Part model, mm, in its own coordinate system. Face numbers are marked on the shaded views. A direction names the side the tool comes from. Coordinates: 2 decimals unless noted, no trailing zeros. Loops run counter-clockwise (first coordinate to the right, second up) from the corner with the lowest first, then second, coordinate; pieces in that order, holes last.
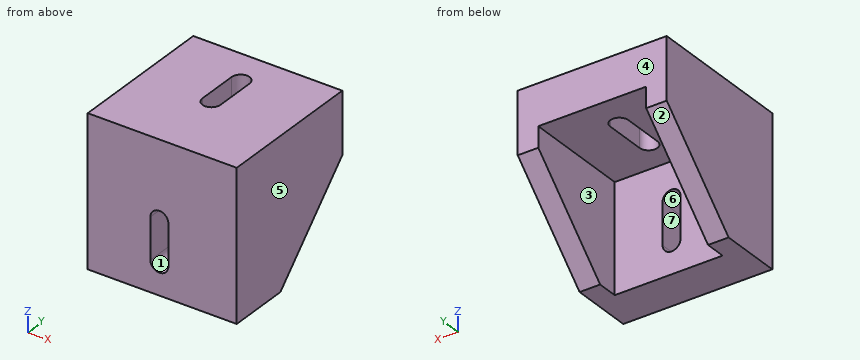
```python
from build123d import *

# Parameters (mm, degrees)
BASE_PLATE_SKETCH_W    = 29
BASE_PLATE_SKETCH_H    = 29
BASE_PLATE_8MM_DEPTH   = 8
BASE_SLOT_3_5MM_DEPTH  = 8
UPRIGHT_WALL_SKETCH_W  = 29
UPRIGHT_WALL_SKETCH_H  = 21
UPRIGHT_WALL_8MM_DEPTH = 8
WALL_SLOT_3_5MM_DEPTH  = 8
SIDE_BOSS_A_4MM_DEPTH  = 4
SIDE_BOSS_B_4MM_DEPTH  = 4


with BuildPart() as part:
    # Base Plate Sketch → Base Plate 8mm (new body)
    with BuildSketch(Plane.XY):
        with Locations((14.5, 14.5)):
            Rectangle(BASE_PLATE_SKETCH_W, BASE_PLATE_SKETCH_H)
    extrude(amount=BASE_PLATE_8MM_DEPTH)

    # Base Slot Sketch → Base Slot 3.5mm (cut)
    with BuildSketch(Plane.XY.offset(8)):
        with BuildLine():
            Line((12.234144505, 22.262653084), (12.234144505, 14.262653084))
            ThreePointArc((12.234144505, 14.262653084), (13.984144505, 12.512653084), (15.734144505, 14.262653084))
            Line((15.734144505, 14.262653084), (15.734144505, 22.262653084))
            ThreePointArc((15.734144505, 22.262653084), (13.984144505, 24.012653084), (12.234144505, 22.262653084))
        make_face()
    extrude(amount=-BASE_SLOT_3_5MM_DEPTH, mode=Mode.SUBTRACT)

    # Upright Wall Sketch → Upright Wall 8mm (add)
    with BuildSketch(Plane.XZ):
        with Locations((14.5, -10.5)):
            Rectangle(UPRIGHT_WALL_SKETCH_W, UPRIGHT_WALL_SKETCH_H)
    extrude(amount=-UPRIGHT_WALL_8MM_DEPTH)

    # Wall Slot Sketch → Wall Slot 3.5mm (cut)
    with BuildSketch(Plane(origin=(0, 8, 0), x_dir=(1, 0, 0), z_dir=(0, 1, 0))):
        with BuildLine():
            Line((12.192184218, 15), (12.192184218, 7))
            ThreePointArc((12.192184218, 7), (13.942184218, 5.25), (15.692184218, 7))
            Line((15.692184218, 7), (15.692184218, 15))
            ThreePointArc((15.692184218, 15), (13.942184218, 16.75), (12.192184218, 15))
        make_face()
    extrude(amount=-WALL_SLOT_3_5MM_DEPTH, mode=Mode.SUBTRACT)

    # Side Boss A Sketch → Side Boss A 4mm (add)
    with BuildSketch(Plane(origin=(29, 0, 0), x_dir=(0, 0, -1), z_dir=(1, 0, 0))):
        Polygon((0, 29), (4, 29), (21, 12), (21, 8), (0, 8), align=None)
    extrude(amount=-SIDE_BOSS_A_4MM_DEPTH)

    # Side Boss B Sketch → Side Boss B 4mm (add)
    with BuildSketch(Plane.ZY):
        Polygon((0, 29), (-4, 29), (-21, 12), (-21, 8), (0, 8), align=None)
    extrude(amount=-SIDE_BOSS_B_4MM_DEPTH)


solid = part.part
```
Q1. Probe line 1 (X direction, y = 2.75, z = -10.5); line 2 (X direction, y = 14.5, z = -15); line 3 (Z direction, x = 23.5, y = 22). List the from-to ranges inside material, lowest first.
Q2. Saw through at A-A (z = -14). List the corners of the cut face in (x, y).
Q3. Saw through at B-B (y = 17). List the corners of the cut face in (x, z), plus the area to 3 significant figures.
Q4. Saw through at D-D (x = 12.75). List the corners of the cut face in (y, z), plus the area to 3 significant figures.
Q5. Tool access for the marked faces 1, 2 and 3: list every direction of +Z, -Z, +X, -X, +Y, -Y with a clear straight run to the whole face (end or side of a thin tool).
Q6. Drop flat-ended pins along their axis: P1, Ø5, axis at x = 16, y = 24.5, coming from the -Z side; P2, Ø4, axis at x = 21.5, z = -13.5, coming from the +Y side. Give the stop position or say it passes through.
Q7. Mould opens along X. For the marked faces 4, 5, 6 and 7 say: released by +X, released by -X, zero draft, split by the parting line, or undercut.
Q8. Saw through at C-C (z = 0.75). List the corners of the cut face in (x, y).
Checked values:
1. line 1: x = 0 to 12.19, 15.69 to 29
1. line 2: x = 0 to 4, 25 to 29
1. line 3: z = 0 to 8
2. outline: (0, 0) - (12.19, 0) - (12.19, 8) - (4, 8) - (4, 19) - (0, 19) - close; (15.69, 0) - (29, 0) - (29, 19) - (25, 19) - (25, 8) - (15.69, 8) - close
3. outline: (0, -16) - (4, -16) - (4, 0) - (12.23, 0) - (12.23, 8) - (0, 8) - close; (15.73, 0) - (25, 0) - (25, -16) - (29, -16) - (29, 8) - (15.73, 8) - close
3. area: 332 mm2
4. outline: (0, -21) - (8, -21) - (8, -16.28) - (0, -16.28) - close; (0, -5.72) - (8, -5.72) - (8, 0) - (13.02, 0) - (13.02, 8) - (0, 8) - close; (23.5, 0) - (29, 0) - (29, 8) - (23.5, 8) - close
4. area: 232 mm2
5. face 1: +Y, -Y
5. face 2: -Z, +X, -X, +Y
5. face 3: -Z, +Y
6. P1: stops at z = 0
6. P2: stops at y = 8
7. face 4: zero draft
7. face 5: released by +X
7. face 6: undercut
7. face 7: undercut
8. outline: (0, 0) - (29, 0) - (29, 29) - (0, 29) - close; hole (12.23, 14.26) arc R1.75 ccw to (15.73, 14.26) - (15.73, 22.26) arc R1.75 ccw to (12.23, 22.26) - close
